Design review of the part built by this model. Coordinates are the model's own, in mm. Coordinates: 2 decimals unless noted, no trailing zeros. Order: outer loops, then holes, each group sorted by start corner. A loop starts at its lowest first (then second) coordinate and runs counter-clockwise, first axis right, second up. Notation, with made-up numbers: M 38,1 L 71,1 A11 ccw 71,21 Z; hole C -14.5,57.25 d11. An arc over 180 degrees is marked long. Use CSV: the item, a comma, the result in double quotes.
```python
from build123d import *

# Parameters (mm, degrees)
SKETCH_2_R          = 2.1
CUT_EXTRUDE_1_DEPTH = 63.197266821


with BuildPart() as part:
    # 草图1 → 旋转1 (revolve)
    with BuildSketch(Plane(origin=(0, 0, 0), x_dir=(1, 0, 0), z_dir=(0, 1, 0)), mode=Mode.PRIVATE) as revolve_1_sk:
        Polygon((-5, 29), (-5, 32.5), (-8, 32.5), (-8, 42.5), (8, 42.5), (8, 32.5), (5, 32.5), (5, 29), align=None)
    revolve(revolve_1_sk.sketch.rotate(Axis((-880.62625216, 0, 0), (1, 0, 0)), 180), axis=Axis((-880.62625216, 0, 0), (1, 0, 0)))

    # 草图2 → 切除-拉伸1 (cut, through all)
    with BuildSketch(Plane(origin=(8, 0, 0), x_dir=(0, 0, -1), z_dir=(1, 0, 0))):
        with Locations((0, 37.5)):
            Circle(SKETCH_2_R)
        with Locations((26.516504294, 26.516504294)):
            Circle(SKETCH_2_R)
        with Locations((37.5, 0)):
            Circle(SKETCH_2_R)
        with Locations((26.516504294, -26.516504294)):
            Circle(SKETCH_2_R)
        with Locations((0, -37.5)):
            Circle(SKETCH_2_R)
        with Locations((-26.516504294, -26.516504294)):
            Circle(SKETCH_2_R)
        with Locations((-37.5, 0)):
            Circle(SKETCH_2_R)
        with Locations((-26.516504294, 26.516504294)):
            Circle(SKETCH_2_R)
        with BuildLine():
            ThreePointArc((20.899942589, 34.105606574), (15.307337295, 36.9551813), (9.337814554, 38.894796816))
            ThreePointArc((9.337814554, 38.894796816), (6.323276344, 37.047485425), (8.170587735, 34.032947214))
            ThreePointArc((8.170587735, 34.032947214), (13.393920133, 32.335783638), (18.287449765, 29.842405752))
            ThreePointArc((18.287449765, 29.842405752), (21.725296588, 30.667759751), (20.899942589, 34.105606574))
        make_face()
        with BuildLine():
            ThreePointArc((38.894796816, 9.337814554), (36.9551813, 15.307337295), (34.105606574, 20.899942589))
            ThreePointArc((34.105606574, 20.899942589), (30.667759751, 21.725296588), (29.842405752, 18.287449765))
            ThreePointArc((29.842405752, 18.287449765), (32.335783638, 13.393920133), (34.032947214, 8.170587735))
            ThreePointArc((34.032947214, 8.170587735), (37.047485425, 6.323276344), (38.894796816, 9.337814554))
        make_face()
        with BuildLine():
            ThreePointArc((34.105606574, -20.899942589), (36.9551813, -15.307337295), (38.894796816, -9.337814554))
            ThreePointArc((38.894796816, -9.337814554), (37.047485425, -6.323276344), (34.032947214, -8.170587735))
            ThreePointArc((34.032947214, -8.170587735), (32.335783638, -13.393920133), (29.842405752, -18.287449765))
            ThreePointArc((29.842405752, -18.287449765), (30.667759751, -21.725296588), (34.105606574, -20.899942589))
        make_face()
        with BuildLine():
            ThreePointArc((9.337814554, -38.894796816), (15.307337295, -36.9551813), (20.899942589, -34.105606574))
            ThreePointArc((20.899942589, -34.105606574), (21.725296588, -30.667759751), (18.287449765, -29.842405752))
            ThreePointArc((18.287449765, -29.842405752), (13.393920133, -32.335783638), (8.170587735, -34.032947214))
            ThreePointArc((8.170587735, -34.032947214), (6.323276344, -37.047485425), (9.337814554, -38.894796816))
        make_face()
        with BuildLine():
            ThreePointArc((-20.899942589, -34.105606574), (-15.307337295, -36.9551813), (-9.337814554, -38.894796816))
            ThreePointArc((-9.337814554, -38.894796816), (-6.323276344, -37.047485425), (-8.170587735, -34.032947214))
            ThreePointArc((-8.170587735, -34.032947214), (-13.393920133, -32.335783638), (-18.287449765, -29.842405752))
            ThreePointArc((-18.287449765, -29.842405752), (-21.725296588, -30.667759751), (-20.899942589, -34.105606574))
        make_face()
        with BuildLine():
            ThreePointArc((-38.894796816, -9.337814554), (-36.9551813, -15.307337295), (-34.105606574, -20.899942589))
            ThreePointArc((-34.105606574, -20.899942589), (-30.667759751, -21.725296588), (-29.842405752, -18.287449765))
            ThreePointArc((-29.842405752, -18.287449765), (-32.335783638, -13.393920133), (-34.032947214, -8.170587735))
            ThreePointArc((-34.032947214, -8.170587735), (-37.047485425, -6.323276344), (-38.894796816, -9.337814554))
        make_face()
        with BuildLine():
            ThreePointArc((-34.105606574, 20.899942589), (-36.9551813, 15.307337295), (-38.894796816, 9.337814554))
            ThreePointArc((-38.894796816, 9.337814554), (-37.047485425, 6.323276344), (-34.032947214, 8.170587735))
            ThreePointArc((-34.032947214, 8.170587735), (-32.335783638, 13.393920133), (-29.842405752, 18.287449765))
            ThreePointArc((-29.842405752, 18.287449765), (-30.667759751, 21.725296588), (-34.105606574, 20.899942589))
        make_face()
        with BuildLine():
            ThreePointArc((-9.337814554, 38.894796816), (-15.307337295, 36.9551813), (-20.899942589, 34.105606574))
            ThreePointArc((-20.899942589, 34.105606574), (-21.725296588, 30.667759751), (-18.287449765, 29.842405752))
            ThreePointArc((-18.287449765, 29.842405752), (-13.393920133, 32.335783638), (-8.170587735, 34.032947214))
            ThreePointArc((-8.170587735, 34.032947214), (-6.323276344, 37.047485425), (-9.337814554, 38.894796816))
        make_face()
    extrude(amount=-CUT_EXTRUDE_1_DEPTH, mode=Mode.SUBTRACT)


solid = part.part
```
(1) Add section A-A on y = 0. State the section outline as (x, z) points, and give its area (3 significant figures).
The answers:
outline,"M -8,-42.5 L 8,-42.5 L 8,-39.6 L -8,-39.6 Z; M -8,-35.4 L 8,-35.4 L 8,-32.5 L 5,-32.5 L 5,-29 L -5,-29 L -5,-32.5 L -8,-32.5 Z; M -8,32.5 L -5,32.5 L -5,29 L 5,29 L 5,32.5 L 8,32.5 L 8,35.4 L -8,35.4 Z; M -8,39.6 L 8,39.6 L 8,42.5 L -8,42.5 Z"
area,"256 mm2"
(2) Add section D-D on z = -37.5. State the section outline as (x, y) points, and give its area (3 significant figures).
The answers:
outline,"M -8,-20 L 8,-20 L 8,-13.92 L -8,-13.92 Z; M -8,-6.48 L 8,-6.48 L 8,-2.1 L -8,-2.1 Z; M -8,2.1 L 8,2.1 L 8,6.48 L -8,6.48 Z; M -8,13.92 L 8,13.92 L 8,20 L -8,20 Z"
area,"335 mm2"
(3) Clearance check with flat-ended pins moving along their axes: P1, Ø2, axis at x = 0, y = 20, coming from the +Z side; P2, Ø2, axis at x = -2.5, z = -4.5, coming from the -Y side; P3, Ø6, axis at x = -5.5, z = 2.5, coming from the -Y side. State where each tip first meets the part, or that it passes through.
The answers:
P1,"stops at z = 38.02"
P2,"stops at y = -42.36"
P3,"stops at y = -42.5"
(4) The part is to be moulded in two halves that separate along Y. For faces 1 (the face through (6.48, -9.76, 31)), 2 (the face through (0.11, 36.92, -15.39)), 3 (the face through (8, 9, -32)), 4 (the face through (0.112, -12.766, 40.537)), say which applies: pulls with the +Y half, pulls with the -Y half, needs draft (parallel to the pull), parting line crosses it, or undercut.
The answers:
face 1,"undercut"
face 2,"undercut"
face 3,"needs draft"
face 4,"parting line crosses it"
(5) Add section C-C on y = -31.5. State the section outline as (x, z) points.
The answers:
outline,"M -8,-28.53 L 8,-28.53 L 8,-22.05 L -8,-22.05 Z; M -8,-15.26 L 8,-15.26 L 8,-8 L 5,-8 L 5,8 L 8,8 L 8,15.26 L -8,15.26 L -8,8 L -5,8 L -5,-8 L -8,-8 Z; M -8,22.05 L 8,22.05 L 8,28.53 L -8,28.53 Z"
(6) Wall thickness on probe 1 along Y at (x, z) = (-2, 0); probe 2 along Y at (x, z) = (-0.5, -9); probe 3 along Z at (x, y) = (7.25, -20): over which ranges is each line inside the solid? List them lowest first.
The answers:
probe 1,"y = -42.5 to -39.6, -35.4 to -29, 29 to 35.4, 39.6 to 42.5"
probe 2,"y = -41.54 to -38.95, -33.82 to -27.57, 27.57 to 33.82, 38.95 to 41.54"
probe 3,"z = -37.5 to -34.64, -29.51 to -25.62, 25.62 to 29.51, 34.64 to 37.5"
